Input: part model. Units: mm. Frame: model coordinates. A direction names the side the tool comes from. Round coordinates to 2 decimals unless told otherwise and drop trailing zeros. Write each loop counter-clockwise with the first axis right and the second up, starting at its lowest first coordinate (ties: lowest second). Pieces come first, ordered by that corner, then holes. Notation, with made-up numbers: (-1, 0) -> (15, 0) arc R13 cw to (15, 19) -> close; hole circle Ø8 at (47.25, 15.5). An arc over 180 degrees is marked (long way). Use CSV: the item, a comma, the result in double quotes.
```python
from build123d import *

# Parameters (mm, degrees)
BOSS_EXTRUDE1_DEPTH = 6
SKETCH3_R           = 9
BOSS_EXTRUDE2_DEPTH = 32
SKETCH5_R           = 3.674588618
CUT_EXTRUDE1_DEPTH  = 12


with BuildPart() as part:
    # Sketch2 → Boss-Extrude1 (new, symmetric)
    with BuildSketch(Plane(origin=(0, 0, 10.607757446), x_dir=(-1, 0, 0), z_dir=(0, 0, -1))):
        with BuildLine():
            Line((20.800074125, -16.288280471), (20.800074125, -23.215326818))
            Line((20.800074125, -23.215326818), (33.57764138, -23.215326818))
            Line((33.57764138, -23.215326818), (33.57764138, -16.288280471))
            ThreePointArc((33.57764138, -16.288280471), (27.188857752, -9.899496844), (20.800074125, -16.288280471))
        make_face()
    extrude(amount=BOSS_EXTRUDE1_DEPTH, both=True)

    # Sketch3 → Boss-Extrude2 (add)
    with BuildSketch(Plane.XZ.offset(23.215326818)):
        with Locations(Location((-27.188857752, 10.607757446, 0), (0, 0, 270))):
            Circle(SKETCH3_R)
    extrude(amount=BOSS_EXTRUDE2_DEPTH)

    # Sketch5 → Cut-Extrude1 (cut)
    with BuildSketch(Plane(origin=(0, 0, 4.607757446), x_dir=(-1, 0, 0), z_dir=(0, 0, -1))):
        with Locations((27.188857752, -16.288280471)):
            Circle(SKETCH5_R)
    extrude(amount=-CUT_EXTRUDE1_DEPTH, mode=Mode.SUBTRACT)


solid = part.part
```
Item 1: Pull-direction query (Y, two-part tool) for faces 4 (the face through (-27.3, -9.9, 10.5)), 5 (the face through (-27, -55.215, 11)), 6 (the face through (-24.481, -13.805, 10.524)); classes: +Y half, -Y half, draft (parallel to the pull), parting line (faces both ways), or undercut.
Worked answers:
face 4,"+Y half"
face 5,"-Y half"
face 6,"undercut"
Item 2: Section query A-A on x = -24.75. Return the cut outline in (y, z).
Worked answers:
outline,"(-55.22, 1.94) -> (-23.22, 1.94) -> (-23.22, 4.61) -> (-19.04, 4.61) -> (-19.04, 16.61) -> (-23.22, 16.61) -> (-23.22, 19.27) -> (-55.22, 19.27) -> close; (-13.54, 4.61) -> (-10.38, 4.61) -> (-10.38, 16.61) -> (-13.54, 16.61) -> close"
Item 3: Section query C-C on x = -22.75. Return the cut outline in (y, z).
Worked answers:
outline,"(-55.22, 2.78) -> (-23.22, 2.78) -> (-23.22, 4.61) -> (-11.69, 4.61) -> (-11.69, 16.61) -> (-23.22, 16.61) -> (-23.22, 18.44) -> (-55.22, 18.44) -> close"
Item 4: Section query B-B on z = 14.5. Return the cut outline in (x, y), plus the area to 3 significant figures.
Worked answers:
outline,"(-35.3, -55.22) -> (-19.07, -55.22) -> (-19.07, -23.22) -> (-20.8, -23.22) -> (-20.8, -16.29) arc R6.39 ccw to (-33.58, -16.29) -> (-33.58, -23.22) -> (-35.3, -23.22) -> close; hole circle Ø7.35 at (-27.19, -16.29)"
area,"630 mm²"
Item 5: First-contact query: pin 1 Ø4 at (x, y) = (-24, -17.5) entering from +Z; pin 2 Ø7.5 at (y, z) = (-19, 12) entering from -X; pin 3 Ø5 at (x, y) = (-22.5, -41.5) entering from -Z. Flat tips, straight axial feed; report the tip coordinate or a pass-through.
Worked answers:
pin 1,"stops at z = 16.61"
pin 2,"stops at x = -33.58"
pin 3,"stops at z = 1.88"
Item 6: Set-up query: faces 1 (the face through (-33.578, -20, 11)), 2 (the face through (-30, -19, 16.608)), 3 (the face through (-20.8, -20, 11)). Return all of +Z, -Z, +X, -X, +Y, -Y with unobstructed straight access to the full face (end or side cutting, diameter ignored); none if empty.
Worked answers:
face 1,"+Z, -Z, -X, +Y"
face 2,"+Z, +X, -X, +Y"
face 3,"+Z, -Z, +X, +Y"
Item 7: Line query: line 1 (Y direction, x = -20, z = 8.25); line 2 (Z direction, x = -23, y = -21); line 3 (X direction, y = -13.5, z = 11). Output: solid intervals per line, ascending.
Worked answers:
line 1,"y = -55.22 to -23.22"
line 2,"z = 4.61 to 16.61"
line 3,"x = -32.94 to -29.58, -24.8 to -21.44"
Item 8: Section query D-D on z = 9.5. Return the cut outline in (x, y), plus the area to 3 significant figures.
Worked answers:
outline,"(-36.12, -55.22) -> (-18.26, -55.22) -> (-18.26, -23.22) -> (-20.8, -23.22) -> (-20.8, -16.29) arc R6.39 ccw to (-33.58, -16.29) -> (-33.58, -23.22) -> (-36.12, -23.22) -> close; hole circle Ø7.35 at (-27.19, -16.29)"
area,"682 mm²"
